from build123d import *

# Parameters (mm, degrees)
SKETCH_1_W                  = 100
SKETCH_1_H                  = 90
EXTRUDE_1_DEPTH             = 7.5
HOLE_WIZARD_M6_1_D          = 5
HOLE_WIZARD_M6_1_DEPTH      = 15
HOLE_WIZARD_M6_1_TIP        = 1.502151548
CUT_EXTRUDE_1_DEPTH         = 5
CUT_EXTRUDE_2_DEPTH         = 69.007352544
PATTERN_LINEAR_1_COUNT      = 2
PATTERN_LINEAR_1_PITCH      = 34
PATTERN_LINEAR_1_COUNT_DIR2 = 2
PATTERN_LINEAR_1_PITCH_DIR2 = 44
CHAMFER_1_SIZE              = 2


with BuildPart() as part:
    # 草图1 → 凸台-拉伸1 (new, symmetric)
    with BuildSketch(Plane.XY):
        Rectangle(SKETCH_1_W, SKETCH_1_H)
    extrude(amount=EXTRUDE_1_DEPTH, both=True)

    # M6 螺纹孔1
    with Locations(Plane.ZY.offset(50)):
        with Locations((0, 35), (0, 0), (0, -35)):
            Hole(HOLE_WIZARD_M6_1_D / 2, depth=HOLE_WIZARD_M6_1_DEPTH)
            with Locations((0, 0, -(HOLE_WIZARD_M6_1_DEPTH + HOLE_WIZARD_M6_1_TIP / 2))):  # 118° drill point
                Cone(0, HOLE_WIZARD_M6_1_D / 2, HOLE_WIZARD_M6_1_TIP, mode=Mode.SUBTRACT)

    # 草图4 → 切除-拉伸1 (cut)
    with BuildSketch(Plane.XY.offset(7.5)):
        with BuildLine():
            Line((14.5, -23), (14.5, -33))
            ThreePointArc((14.5, -33), (8, -39.5), (1.5, -33))
            Line((1.5, -33), (1.5, -23))
            ThreePointArc((1.5, -23), (8, -16.5), (14.5, -23))
        make_face()
    cut_extrude_1 = extrude(amount=-CUT_EXTRUDE_1_DEPTH, mode=Mode.SUBTRACT)

    # 草图5 → 切除-拉伸2 (cut, through all)
    with BuildSketch(Plane.XY.offset(2.5)):
        with BuildLine():
            Line((5, -23), (5, -33))
            ThreePointArc((5, -33), (8, -36), (11, -33))
            Line((11, -33), (11, -23))
            ThreePointArc((11, -23), (8, -20), (5, -23))
        make_face()
    cut_extrude_2 = extrude(amount=-CUT_EXTRUDE_2_DEPTH, mode=Mode.SUBTRACT)

    # 阵列(线性)1: 切除-拉伸1, Cut-Extrude 2 2 × 2
    with Locations(*[(i * PATTERN_LINEAR_1_PITCH, j * PATTERN_LINEAR_1_PITCH_DIR2, 0) for i in range(PATTERN_LINEAR_1_COUNT) for j in range(PATTERN_LINEAR_1_COUNT_DIR2) if (i, j) != (0, 0)]):
        add(cut_extrude_1, mode=Mode.SUBTRACT)
        add(cut_extrude_2, mode=Mode.SUBTRACT)

    # 倒角1
    chamfer_1_edges = [part.edges().sort_by_distance(p)[0] for p in [
        (50, -45, 0),
        (-50, -45, 0),
        (-50, 45, 0),
        (50, 45, 0),
    ]]
    chamfer(chamfer_1_edges, length=CHAMFER_1_SIZE)


solid = part.part
Here's how the part is built. I have some questions about the finished solid (model axes, mm). A direction names the side the tool comes from. Coordinates: 2 decimals unless noted, no trailing zeros. Order: outer loops, then holes, each group sorted by start corner. A loop starts at its lowest first (then second) coordinate and runs counter-clockwise, first axis right, second up.
Item 1: For faces 4 (the face through (41.9, 27.5, 5)), 5 (the face through (-42.4, -32.89, -1.34)), 6 (the face through (42, 24, -2)), which set-ups out of +Z, -Z, +X, -X, +Y, -Y let a thin tool reach every point of the face, with its end or its side?
Result sheet:
face 4: +Z
face 5: -X
face 6: +Z, -Z
Item 2: If we section it at B-B on x = 42: List the corners of the cut face in (y, z) for me, plus the area to 3 significant figures.
Result sheet:
outline: (-45, -7.5) - (-36, -7.5) - (-36, 2.5) - (-39.5, 2.5) - (-39.5, 7.5) - (-45, 7.5) - close; (-20, -7.5) - (8, -7.5) - (8, 2.5) - (4.5, 2.5) - (4.5, 7.5) - (-16.5, 7.5) - (-16.5, 2.5) - (-20, 2.5) - close; (24, -7.5) - (45, -7.5) - (45, 7.5) - (27.5, 7.5) - (27.5, 2.5) - (24, 2.5) - close
area: 800 mm2
Item 3: If we mould it in two halves opening along Z, with no side actions, what happens to faces 1 (the face through (39, 16, -2)), 2 (the face through (-33.76, 35.43, -0.06)), 3 (the face through (38, -28, 2.5))? For each: +Z half, -Z half, draft (parallel to the pull), parting line (faces both ways), or undercut.
Result sheet:
face 1: draft
face 2: undercut
face 3: +Z half
Item 4: For P1, Ø3, axis at y = 0, z = 0, coming from the -X side, with a flat end and sliding along its axis, tell me the tip position at first contact or that it passes through.
Result sheet:
P1: stops at x = -34.4
Item 5: If we section it at C-C on z = -4.75: List the corners of the cut face in (x, y) for me.
Result sheet:
outline: (-50, -43) - (-48, -45) - (48, -45) - (50, -43) - (50, 43) - (48, 45) - (-48, 45) - (-50, 43) - close; hole (5, -33) arc R3 ccw to (11, -33) - (11, -23) arc R3 ccw to (5, -23) - close; hole (5, 11) arc R3 ccw to (11, 11) - (11, 21) arc R3 ccw to (5, 21) - close; hole (39, -33) arc R3 ccw to (45, -33) - (45, -23) arc R3 ccw to (39, -23) - close; hole (39, 11) arc R3 ccw to (45, 11) - (45, 21) arc R3 ccw to (39, 21) - close
Item 6: If we section it at A-A on y = -28: List the corners of the cut face in (x, z) for me.
Result sheet:
outline: (-50, -7.5) - (5, -7.5) - (5, 2.5) - (1.5, 2.5) - (1.5, 7.5) - (-50, 7.5) - close; (11, -7.5) - (39, -7.5) - (39, 2.5) - (35.5, 2.5) - (35.5, 7.5) - (14.5, 7.5) - (14.5, 2.5) - (11, 2.5) - close; (45, -7.5) - (50, -7.5) - (50, 7.5) - (48.5, 7.5) - (48.5, 2.5) - (45, 2.5) - close
Item 7: If we section it at D-D on y = 6: List the corners of the cut face in (x, z) for me.
Result sheet:
outline: (-50, -7.5) - (50, -7.5) - (50, 7.5) - (46.15, 7.5) - (46.15, 2.5) - (37.85, 2.5) - (37.85, 7.5) - (12.15, 7.5) - (12.15, 2.5) - (3.85, 2.5) - (3.85, 7.5) - (-50, 7.5) - close
Item 8: I need wall thicknesses on line 1 (Y direction, x = -47, z = 0); line 2 (X direction, y = 15, z = 7.25); line 3 (X direction, y = 13, z = -4.25). Which ranges of each line are inside material? Lowest first, please.
Result sheet:
line 1: y = -45 to -37.5, -32.5 to -2.5, 2.5 to 32.5, 37.5 to 45
line 2: x = -50 to 1.5, 14.5 to 35.5, 48.5 to 50
line 3: x = -50 to 5, 11 to 39, 45 to 50
